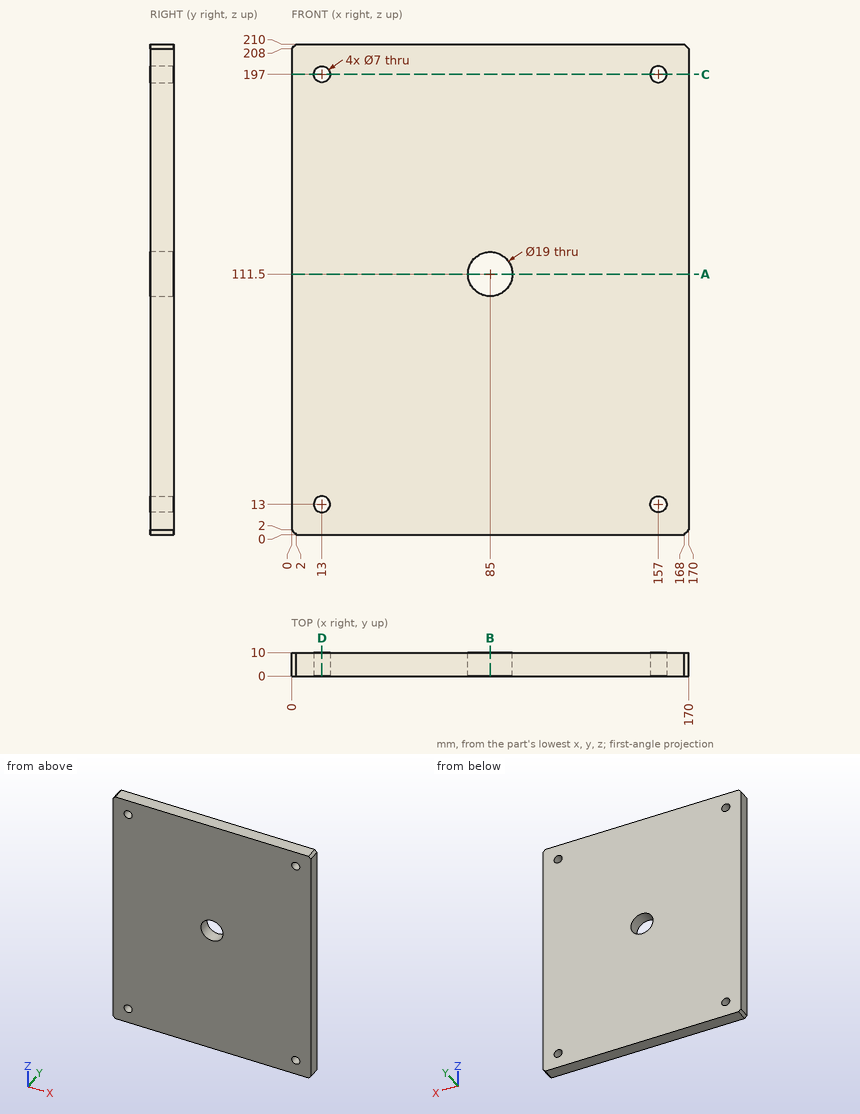
Answer from the drawing. Dimensions are ordinates in mm from the lowest x, y and z of the part. Give positions to 0.01 mm unless a question says otherwise; leave off trailing zeros. Order: outer loops, then holes, each group sorted by start corner. A loop starts at its lowest first (then second) coordinate and runs counter-clockwise, first axis right, second up.
(1) Given pin 1 (4 mm diameter, centred on x = 13, z = 13, fed in from +Y); pin 2 (1.5 mm diameter, centred on x = 104, z = 153, fed in from -Y), each flat-ended and moving along its own axis, determine where each tip first touches the part or whether it passes through.
(2) Find section B-B (x = 85). Give the vertices of the cut face in (y, z), plus the area to 3 significant figures.
(3) Find section C-C (z = 197). Give the vertices of the cut face in (x, y).
(4) Straight lines are drawn through the part: L1, parallel to X at y = 3.5, z = 197; L2, parallel to Z at x = 13, y = 6.25; L3, parallel to X at y = 7, z = 111.5. For each, find the intervals that lie inside material, in ascending order.
(5) Find section D-D (x = 13). Give the vertices of the cut face in (y, z), plus the area to 3 significant figures.
(6) Find section A-A (z = 111.5). Give the vertices of the cut face in (x, y).
Result sheet:
1. pin 1: passes through
1. pin 2: stops at y = 0
2. outline: (0, 0) - (10, 0) - (10, 102) - (0, 102) - close; (0, 121) - (10, 121) - (10, 210) - (0, 210) - close
2. area: 1,910 mm2
3. outline: (0, 0) - (9.5, 0) - (9.5, 10) - (0, 10) - close; (16.5, 0) - (153.5, 0) - (153.5, 10) - (16.5, 10) - close; (160.5, 0) - (170, 0) - (170, 10) - (160.5, 10) - close
4. L1: x = 0 to 9.5, 16.5 to 153.5, 160.5 to 170
4. L2: z = 0 to 9.5, 16.5 to 193.5, 200.5 to 210
4. L3: x = 0 to 75.5, 94.5 to 170
5. outline: (0, 0) - (10, 0) - (10, 9.5) - (0, 9.5) - close; (0, 16.5) - (10, 16.5) - (10, 193.5) - (0, 193.5) - close; (0, 200.5) - (10, 200.5) - (10, 210) - (0, 210) - close
5. area: 1,960 mm2
6. outline: (0, 0) - (75.5, 0) - (75.5, 10) - (0, 10) - close; (94.5, 0) - (170, 0) - (170, 10) - (94.5, 10) - close
